Could you check a few things on this model? Use its own coordinates, in mm. A direction names the side the tool comes from. Give positions to 0.01 mm unless a question says otherwise; leave off trailing zeros. Loops run counter-clockwise (first coordinate to the right, second up) from the corner with the lowest first, then second, coordinate; pieces in that order, holes last. Notation, with made-up numbers: (42, -4) - (97, -4) arc R14 cw to (97, 1) - close; hole circle Ø2 at (39, 16). An arc over 180 degrees is marked (long way). One line per item, written item: value. Start each with the question number.
Q1. I'm going to push flat-ended pins straight in: P1, Ø10, axis at x = -17, y = 10, coming from the -Z side; P2, Ø2, axis at y = 22, z = 9, coming from the +X side; P3, Ø1.5, axis at x = -17, y = 6.5, coming from the -Z side; P4, Ø5, axis at x = 12.5, z = 7, coming from the +Y side. Where does each tip first touch, or does it pass through?
Q2. I want a section at A-A (x = 0). Please give me the cut outline in (y, z), then the cut area to 3 significant figures.
Q3. If I drill on line 1 (Z direction, x = 0, y = 26.5); line 2 (Y direction, x = -19, z = 7), over which ranges is the centre line in solid material (lowest first)? Write a range as from..to.
Q4. I want a section at C-C (y = 25). Please give me the cut outline in (x, z).
Q5. For faces 4 (the face through (-1.055, 0.493, 23.977)), 5 (the face through (16.856, 19.734, -8.767)), which set-ups out of +Z, -Z, +X, -X, +Y, -Y let a thin tool reach every point of the face, with its end or its side?
Q6. If we mould it in two halves opening along Y, with no side actions, what happens to faces 1 (the face through (-7, 39, -18)), 2 (the face through (-18, 0, -3)), 3 (the face through (-1.055, 39.493, 23.977))? For each: released by +Y, released by -Y, zero draft, split by the parting line, or undercut.
Q7. I want a section at D-D (z = -21). Please give me the cut outline in (x, y), then the cut area to 3 significant figures.
Q8. I want a section at B-B (z = 0). Please give me the cut outline in (x, y), then the cut area to 3 significant figures.
```python
from build123d import *


with BuildPart() as part:
    # Sketch2 → Revolve2 (revolve)
    with BuildSketch(Plane(origin=(0, 0, 0), x_dir=(0, 0, -1), z_dir=(1, 0, 0))):
        Polygon((24, 40), (24, 39), (19, 39), (19, 1), (24, 1), (24, 0), (18, 0), (18, 40), align=None)
    revolve(axis=Axis((0, 0, 0), (0, 1, 0)))


solid = part.part
```
Worked answers:
1. P1: stops at z = -14.73
1. P2: stops at x = 17.23
1. P3: stops at z = -9.85
1. P4: passes through
2. outline: (0, -24) - (1, -24) - (1, -19) - (39, -19) - (39, -24) - (40, -24) - (40, -18) - (0, -18) - close; (0, 18) - (40, 18) - (40, 24) - (39, 24) - (39, 19) - (1, 19) - (1, 24) - (0, 24) - close
2. area: 100 mm²
3. line 1: z = -19..-18, 18..19
3. line 2: y = 0..1, 39..40
4. outline: circle Ø38 at (0, 0); hole circle Ø36 at (0, 0)
5. face 4: +Y, -Y
5. face 5: none
6. face 1: undercut
6. face 2: released by -Y
6. face 3: zero draft
7. outline: (-11.62, 0) - (11.62, 0) - (11.62, 1) - (-11.62, 1) - close; (-11.62, 39) - (11.62, 39) - (11.62, 40) - (-11.62, 40) - close
7. area: 46.5 mm²
8. outline: (-24, 0) - (-18, 0) - (-18, 40) - (-24, 40) - (-24, 39) - (-19, 39) - (-19, 1) - (-24, 1) - close; (18, 0) - (24, 0) - (24, 1) - (19, 1) - (19, 39) - (24, 39) - (24, 40) - (18, 40) - close
8. area: 100 mm²
